The listing builds one solid part. Answer for the finished solid, in the listing's coordinates (mm). A direction names the side the tool comes from. Round coordinates to 2 decimals unless told otherwise and drop trailing zeros. Order: outer loops, then holes, each group sorted by start corner. A loop starts at its lowest first (then second) coordinate and runs counter-clockwise, first axis right, second up. Notation, with made-up numbers: (53, 21.25) - (81, 21.25) arc R20 cw to (81, 44.25) - close; hole circle Ø1 at (-36, 65). An arc over 180 degrees is marked (long way). Use CSV: the item, a comma, the result in double quotes. Start each with the question number.
Item 1: For faces 1 (the conical face through (3.62, -3.12, -5.38)), 2 (the cylindrical face through (-20.9, -0.9, 2.86)), determine the directions among +Z, -Z, +X, -X, +Y, -Y from which every point of the face is accessible in a straight line to the end or side of a thin tool.
Item 2: Straight lines are drawn through the part: line 1 along X through (y, z) = (0.5, 4); line 2 along Y through (x, z) = (-28, -0.5); line 3 along Z through (x, y) = (-22, 1.5). For each, find the intervals that lie inside material, in ascending order. Write a range as [from, to].
Item 3: Flat-ended cylindrical pins translate along their axes: P1, Ø5, axis at x = -39.5, z = -4.5, coming from the +Y side; P2, Ø1.5, axis at x = -32, z = -1, coming from the -Y side; P3, Ø2, axis at x = -21.5, z = -3, coming from the -Y side. Find the tip coordinate at first contact, or state that the pin passes through.
Item 4: Find section A-A, the plane x = -24.5. Give the vertices of the cut face in (y, z).
```python
from build123d import *

# Parameters (mm, degrees)
BOSS_EXTRUDE1_DEPTH = 4
SKETCH2_OUTSIDE_W   = 40.846
SKETCH2_OUTSIDE_H   = 42.702
SKETCH2_OUTSIDE_R   = 6
CUT_EXTRUDE1_DEPTH  = 20
CUT_EXTRUDE1_DRAFT  = -30


with BuildPart() as part:
    # Sketch1 → Boss-Extrude1 (new body)
    with BuildSketch(Plane(origin=(0, 0, 0), x_dir=(0, 0, -1), z_dir=(1, 0, 0))):
        Polygon((0, -6.92820323), (6, -3.464101615), (6, 3.464101615), (0, 6.92820323), (-6, 3.464101615), (-6, -3.464101615), align=None)
    extrude(amount=BOSS_EXTRUDE1_DEPTH)


with BuildPart() as cut_extrude1_tool:
    # Sketch2 outside → Cut-Extrude1 (with draft: the straight prism first)
    with BuildSketch(Plane(origin=(4, 0, 0), x_dir=(0, 0, -1), z_dir=(1, 0, 0))):
        Rectangle(SKETCH2_OUTSIDE_W, SKETCH2_OUTSIDE_H)
        Circle(SKETCH2_OUTSIDE_R, mode=Mode.SUBTRACT)
    extrude(amount=-CUT_EXTRUDE1_DEPTH)
    # Cut-Extrude1: the draft: its side faces are tilted about the plane it starts from
    cut_extrude1_sides = [cut_extrude1_tool.faces().sort_by_distance(p)[0] for p in [
        (-6, -21.351, 0),
        (-6, 0, -20.423),
        (-6, 21.351, 0),
        (-6, 0, 20.423),
        (-6, 0, 6),
    ]]
    draft(cut_extrude1_sides, Plane(origin=(4, 0, 0), x_dir=(0, 0, -1), z_dir=(1, 0, 0)), CUT_EXTRUDE1_DRAFT)


with BuildPart() as part_1:
    add(part.part)

    # Cut-Extrude1: cut by cut_extrude1_tool
    add(cut_extrude1_tool.part, mode=Mode.SUBTRACT)

    # Sketch3 → Revolve1 (revolve)
    with BuildSketch(Plane.XY, mode=Mode.PRIVATE) as revolve1_sk:
        Polygon((0, 0), (0, 3), (-41.230297419, 3), (-47, 0.9), (-47, 0), align=None)
    revolve(revolve1_sk.sketch.rotate(Axis((-32.199358367, 0, 0), (1, 0, 0)), 90), axis=Axis((-32.199358367, 0, 0), (1, 0, 0)))


solid = part_1.part
```
Worked out:
1,face 1,"-Z, +X, -Y"
1,face 2,"-X"
2,line 1,"x = [0, 4]"
2,line 2,"y = [-2.96, 2.96]"
2,line 3,"z = [-2.6, 2.6]"
3,P1,"stops at y = 2.24"
3,P2,"stops at y = -2.99"
3,P3,"stops at y = -2.24"
4,outline,"circle Ø6 at (0, 0)"
